from build123d import *

# Parameters (mm, degrees)
HANDLE_PROFILE_SKETCH_W   = 315
HANDLE_PROFILE_SKETCH_H   = 40
HANDLE_BAR_315X40X5_DEPTH = 5
HANGING_END_SKETCH_R      = 20
ROUNDED_HANGING_END_DEPTH = 5
HEAD_NECK_BOSS_DEPTH      = 5
NECK_TRIM_CUT_R25_DEPTH   = 5
NECK_START                = 5
NECK_FILL_BOSS_A_DEPTH    = 5
NECK_FILL_BOSS_B_DEPTH    = 5
OPEN_START                = -5
OPEN_JAW_HEAD_DEPTH       = 5
HANGING_HOLE_SKETCH_R     = 6
HANGING_HOLE_6_DEPTH      = 15


with BuildPart() as part:
    # Handle Profile Sketch → Handle Bar 315x40x5 (new body)
    with BuildSketch(Plane.XY):
        with Locations((157.5, 20)):
            Rectangle(HANDLE_PROFILE_SKETCH_W, HANDLE_PROFILE_SKETCH_H)
    extrude(amount=HANDLE_BAR_315X40X5_DEPTH)

    # Hanging End Sketch → Rounded Hanging End (add)
    with BuildSketch(Plane.XY.offset(5)):
        with Locations((0, 20)):
            Circle(HANGING_END_SKETCH_R)
    extrude(amount=-ROUNDED_HANGING_END_DEPTH)

    # Neck Profile Sketch → Head Neck Boss (add)
    with BuildSketch(Plane.XY.offset(5)):
        with BuildLine():
            Line((315, 40), (315, 37.5))
            Line((315, 37.5), (348.730549951, 37.5))
            ThreePointArc((348.730549951, 37.5), (316.43745902, 57.972802261), (282.689011157, 40))
            Line((282.689011157, 40), (315, 40))
        make_face()
        with BuildLine():
            Line((348.730549951, 2.5), (315, 2.5))
            Line((315, 2.5), (315, 0))
            Line((315, 0), (282.689011157, 0))
            ThreePointArc((282.689011157, 0), (316.43745902, -17.972802261), (348.730549951, 2.5))
        make_face()
    extrude(amount=-HEAD_NECK_BOSS_DEPTH)

    # Neck Trim Sketch R25 → Neck Trim Cut R25 (cut)
    with BuildSketch(Plane.XY.offset(5)):
        with BuildLine():
            Line((315, 37.5), (315, 2.5))
            ThreePointArc((315, 2.5), (307.853571071, 20), (315, 37.5))
        make_face()
    extrude(amount=-NECK_TRIM_CUT_R25_DEPTH, mode=Mode.SUBTRACT)

    # Neck Fill Sketch A → Neck Fill Boss A (add)
    with BuildSketch(Plane.XY.offset(5).offset(NECK_START)):
        with BuildLine():
            Line((348.730549951, 37.5), (315, 37.5))
            ThreePointArc((315, 37.5), (307.853571071, 20), (315, 2.5))
            Line((315, 2.5), (348.730549951, 2.5))
            ThreePointArc((348.730549951, 2.5), (277, 20), (348.730549951, 37.5))
        make_face()
    extrude(amount=-NECK_FILL_BOSS_A_DEPTH)

    # Neck Fill Sketch B → Neck Fill Boss B (add)
    with BuildSketch(Plane(origin=(0, 0, 0), x_dir=(-1, 0, 0), z_dir=(0, 0, -1))):
        with BuildLine():
            Line((-348.730549951, 37.5), (-315, 37.5))
            ThreePointArc((-315, 37.5), (-307.853571071, 20), (-315, 2.5))
            Line((-315, 2.5), (-348.730549951, 2.5))
            ThreePointArc((-348.730549951, 2.5), (-277, 20), (-348.730549951, 37.5))
        make_face()
    extrude(amount=NECK_FILL_BOSS_B_DEPTH)

    # Jaw Head Sketch → Open Jaw Head (add)
    with BuildSketch(Plane(origin=(0, 0, 0), x_dir=(-1, 0, 0), z_dir=(0, 0, -1)).offset(OPEN_START)):
        with BuildLine():
            Line((-268.913125513, 40), (-282.689011157, 40))
            ThreePointArc((-282.689011157, 40), (-285.697034566, 44.193722673), (-289.245570139, 47.941176471))
            ThreePointArc((-289.245570139, 47.941176471), (-279.827228639, 42.055727726), (-268.913125513, 40))
        make_face()
        with BuildLine():
            Line((-268.913125513, 0), (-282.689011157, 0))
            ThreePointArc((-282.689011157, 0), (-285.697034566, -4.193722673), (-289.245570139, -7.941176471))
            ThreePointArc((-289.245570139, -7.941176471), (-279.827228639, -2.055727726), (-268.913125513, 0))
        make_face()
    extrude(amount=OPEN_JAW_HEAD_DEPTH)

    # Hanging Hole Sketch → Hanging Hole Ø6 (cut)
    with BuildSketch(Plane(origin=(0, 0, 0), x_dir=(-1, 0, 0), z_dir=(0, 0, -1))):
        with Locations((0, 20)):
            Circle(HANGING_HOLE_SKETCH_R)
    extrude(amount=-HANGING_HOLE_6_DEPTH, mode=Mode.SUBTRACT)


solid = part.part
Can you work these out from the model? Positions are in its coordinate system, mm. A direction names the side the tool comes from. Round coordinates to 2 decimals unless told otherwise and drop trailing zeros. Write each loop counter-clockwise with the first axis right and the second up, starting at its lowest first coordinate (ties: lowest second). Pieces come first, ordered by that corner, then holes. Notation, with made-up numbers: M 24,33 L 44,33 A31 cw 44,61 Z; hole C 36.5,45 d6. An arc over 180 degrees is marked long. Use a Markdown table: item, result.
Item 1: If I drill on line 1 along Y through (x, z) = (0, 3.75); line 2 along Z through (x, y) = (47.5, 17); line 3 along Y through (x, z) = (310.5, 2), over which ranges is the centre line in solid material (lowest first)? Write a range as [from, to].
Found:
| item | result |
|---|---|
| line 1 | y = [0, 14], [26, 40] |
| line 2 | z = [0, 5] |
| line 3 | y = [-17.73, 8.81], [31.19, 57.73] |
Item 2: We'd pull the mould along Y, two halves only. Please class faces 3 (the face through (279.97, -2.11, 2.54)), 4 (the face through (279.97, 42.11, 2.54)), 5 (the face through (332, 37.5, 3)): released by +Y, released by -Y, zero draft, split by the parting line, or undercut.
Found:
| item | result |
|---|---|
| face 3 | released by -Y |
| face 4 | released by +Y |
| face 5 | undercut |
Item 3: For pin 1 Ø7.5 at (x, z) = (333, 0.5) entering from -Y; pin 2 Ø2.5 at (x, z) = (199.5, 1.5) entering from +Y; pin 3 Ø6 at (y, z) = (28, 6.5) entering from +X, each with a flat end and sliding along its axis, tell me the tip position at first contact or that it passes through.
Found:
| item | result |
|---|---|
| pin 1 | stops at y = -15.23 |
| pin 2 | stops at y = 40 |
| pin 3 | stops at x = 310.4 |
Item 4: I want a section at C-C (x = 323.5). List the corners of the cut face in (y, z) for me.
Found:
| item | result |
|---|---|
| outline | M -17.04,-5 L 2.5,-5 L 2.5,10 L -17.04,10 Z; M 37.5,-5 L 57.04,-5 L 57.04,10 L 37.5,10 Z |
Item 5: I want a section at A-A (z = 2.75). List the corners of the cut face in (x, y) for me.
Found:
| item | result |
|---|---|
| outline | M 0,0 L 268.91,0 A30 cw 289.25,-7.94 A38 ccw 348.73,2.5 L 315,2.5 A25 cw 315,37.5 L 348.73,37.5 A38 ccw 289.25,47.94 A30 cw 268.91,40 L 0,40 A20 ccw Z; hole C 0,20 d12 |
Item 6: Which directions (+Z, -Z, +X, -X, +Y, -Y) give clear straight access to the entire face, cutting with the end or side of a thin tool? Please do faces 1 (the face through (332, 2.5, 3)), 2 (the face through (-20, 20, 3)).
Found:
| item | result |
|---|---|
| face 1 | +Z, -Z, +X |
| face 2 | +Z, -Z, -X |
Item 7: I want a section at D-D (x = 97.5). List the corners of the cut face in (y, z) for me, and give its area (3 significant figures).
Found:
| item | result |
|---|---|
| outline | M 0,0 L 40,0 L 40,5 L 0,5 Z |
| area | 200 mm2 |
Item 8: I want a section at B-B (y = 20). List the corners of the cut face in (x, z) for me.
Found:
| item | result |
|---|---|
| outline | M -20,0 L -6,0 L -6,5 L -20,5 Z; M 6,0 L 277,0 L 277,-5 L 307.85,-5 L 307.85,10 L 277,10 L 277,5 L 6,5 Z |
